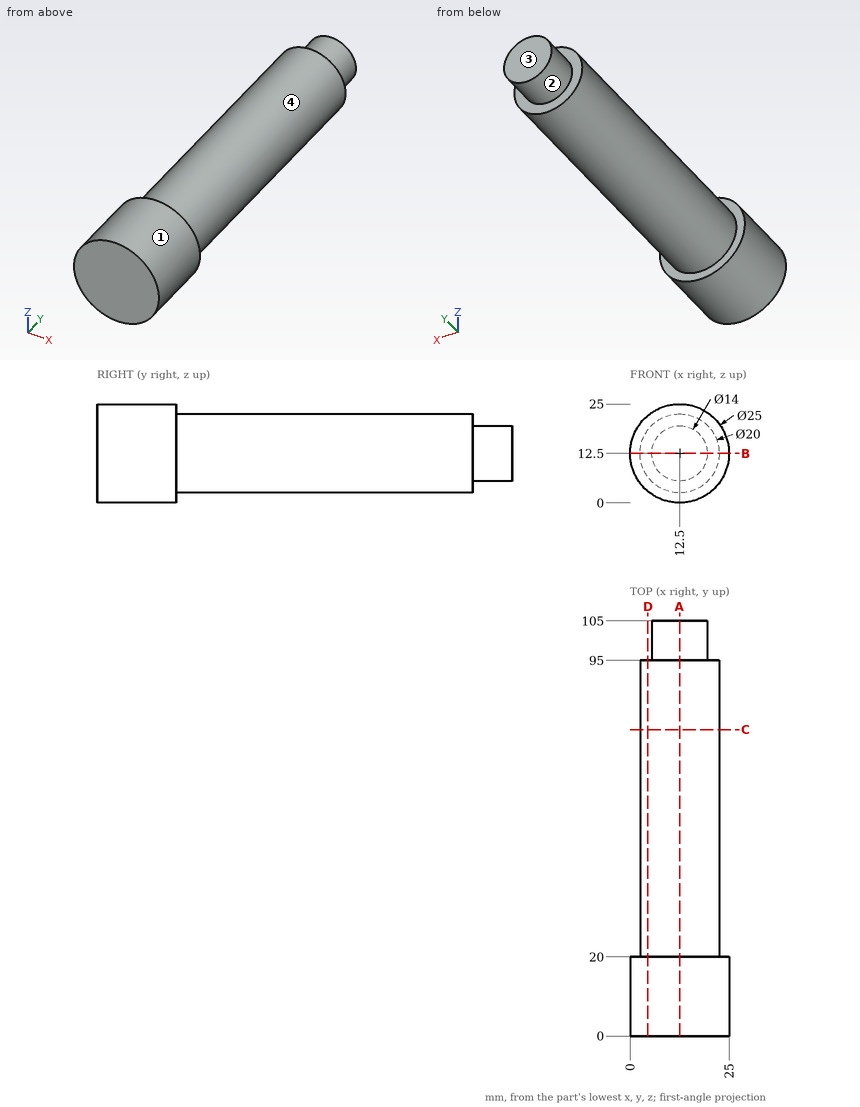
Answer from the drawing. Dimensions are ordinates in mm from the lowest x, y and z of the part. A direction names the side the tool comes from. Round coordinates to 2 decimals unless told otherwise and drop trailing zeros. Write each loop counter-clockwise with the first axis right and the second up, starting at its lowest first coordinate (ties: lowest second). Pieces come first, ordered by that corner, then holes. Notation, with made-up numbers: (-18, 52.5) - (21, 52.5) arc R36 cw to (21, 89.5) - close; hole circle Ø4 at (-34.75, 12.25). An arc over 180 degrees is marked (long way). Use a Markdown table: item, result.
(1) The part is cut by section C-C (y = 77.5). Write down the section's boundary in (x, z).
Reported:
| item | result |
|---|---|
| outline | circle Ø20 at (12.5, 12.5) |
(2) Straight lines are drawn through the part: line 1 along Y through (x, z) = (17.5, 6); line 2 along Y through (x, z) = (2.25, 19.25); line 3 along Z through (x, y) = (13, 19.5). For each, find the intervals that lie inside material, in ascending order. Write a range as [from, to].
Reported:
| item | result |
|---|---|
| line 1 | [0, 95] |
| line 2 | [0, 20] |
| line 3 | [0.01, 24.99] |
(3) The part is cut by section D-D (x = 4.5). Write down the section's boundary in (y, z), then the cut area to 3 significant figures.
Reported:
| item | result |
|---|---|
| outline | (0, 2.9) - (20, 2.9) - (20, 6.5) - (95, 6.5) - (95, 18.5) - (20, 18.5) - (20, 22.1) - (0, 22.1) - close |
| area | 1,280 mm2 |
(4) The part is cut by section A-A (x = 12.5). Write down the section's boundary in (y, z), then the cut area to 3 significant figures.
Reported:
| item | result |
|---|---|
| outline | (0, 0) - (20, 0) - (20, 2.5) - (95, 2.5) - (95, 5.5) - (105, 5.5) - (105, 19.5) - (95, 19.5) - (95, 22.5) - (20, 22.5) - (20, 25) - (0, 25) - close |
| area | 2,140 mm2 |
(5) The part is cut by section B-B (z = 12.5). Write down the section's boundary in (x, y), then the cut area to 3 significant figures.
Reported:
| item | result |
|---|---|
| outline | (0, 0) - (25, 0) - (25, 20) - (22.5, 20) - (22.5, 95) - (19.5, 95) - (19.5, 105) - (5.5, 105) - (5.5, 95) - (2.5, 95) - (2.5, 20) - (0, 20) - close |
| area | 2,140 mm2 |
(6) Which of the six approach directions +Z, -Z, +X, -X, +Y, -Y give full straight-line access (tool end or side, diameter ignored) to the marked faces 1 and 2?
Reported:
| item | result |
|---|---|
| face 1 | +Y, -Y |
| face 2 | +Y |
(7) The mould has two halves that part along Z. Classify the marked faces 3 and 4: released by +Z, released by -Z, zero draft, split by the parting line, or undercut.
Reported:
| item | result |
|---|---|
| face 3 | zero draft |
| face 4 | split by the parting line |
(8) Each of these flat-tipped pins is pushed along its axis until it touches: pin 1 Ø2 at (y, z) = (68.5, 6) entering from -X; pin 2 Ø1.5 at (x, y) = (13.5, 49) entering from -Z; pin 3 Ø4 at (x, z) = (8, 3) entering from +Y. Where does it stop, or does it pass through?
Reported:
| item | result |
|---|---|
| pin 1 | x = 4.15 |
| pin 2 | z = 2.5 |
| pin 3 | y = 95 |
